```python
from build123d import *

# Parameters (mm, degrees)
BOSS_EXTRUDE1_DEPTH = 10


with BuildPart() as part:
    # Sketch1 → Boss-Extrude1 (new body)
    with BuildSketch(Plane.XY):
        with BuildLine():
            Line((-23.745241043, -21.468300121), (26.254758957, -21.468300121))
            ThreePointArc((26.254758957, -21.468300121), (1.254758957, 3.531699879), (-23.745241043, -21.468300121))
        make_face()
    extrude(amount=BOSS_EXTRUDE1_DEPTH)

    # Cut-Sweep1: sweep along a path in Sketch4
    with BuildLine(Plane.XY.offset(5)) as cut_sweep1_path:
        ThreePointArc((26.254758957, -21.468300121), (1.254758957, 3.531699879), (-23.745241043, -21.468300121))
    # Sketch2 → Cut-Sweep1 (sweep, cut)
    with BuildSketch(Plane.XZ.offset(21.468300121)):
        Polygon((26.254758957, 5), (26.254758957, 6.5), (24.754758957, 5), (26.254758957, 3.5), align=None)
    sweep(path=cut_sweep1_path.line, mode=Mode.SUBTRACT)


solid = part.part
```
Verification items for the finished model (mm, model axes). Round coordinates to 2 decimals unless told otherwise and drop trailing zeros. Loops run counter-clockwise (first coordinate to the right, second up) from the corner with the lowest first, then second, coordinate; pieces in that order, holes last. Notation, with made-up numbers: (14, 24.5) -> (18, 24.5) arc R13 ccw to (18, 47.5) -> close; hole circle Ø4 at (80, 82). An arc over 180 degrees is marked (long way). Answer as a JSON object with one key per item and string values.
Q1. Go/stop test with flat-tipped pins: P1, Ø5, axis at y = -7, z = 8, coming from the +X side; P2, Ø6, axis at x = -8.5, z = 3.5, coming from the +Y side; P3, Ø4, axis at x = -13, z = 5.5, coming from the +Y side. Record where each tip stops, or that it passes through.
Data:
{"P1": "stops at x = 23.2", "P2": "stops at y = 2.6", "P3": "stops at y = 0.17"}
Q2. Section check A-A (z = 1.25). Record the boundary of the cut face in (x, y).
Data:
{"outline": "(-23.75, -21.47) -> (26.25, -21.47) arc R25 ccw to start"}
Q3. Draft check along Z on faces 1 (the cylindrical face through (1.804, 3.526, 1.726)), 2 (the conical face through (1.777, 2.286, 4.74)), 3 (the flat face through (1, -12, 0)), 4 (the conical face through (1.777, 2.265, 5.24)). Enter one of: pulls with the +Z half, pulls with the -Z half, needs draft (parallel to the pull), parting line crosses it, or undercut.
Data:
{"face 1": "needs draft", "face 2": "undercut", "face 3": "pulls with the -Z half", "face 4": "undercut"}
Q4. Scan lines: line 1 (X direction, y = -9.75, z = 7.25); line 2 (X direction, y = -7, z = 4.25); line 3 (Y direction, x = 22, z = 9). Record each from-to range of solid material in increasing order. Write a range as from..to.
Data:
{"line 1": "x = -20.83..23.34", "line 2": "x = -18.21..20.72", "line 3": "y = -21.47..-7.52"}
Q5. Section check B-B (z = 6). Record the boundary of the cut face in (x, y).
Data:
{"outline": "(-23.25, -21.47) -> (25.75, -21.47) arc R24.5 ccw to start"}
